Geometry: final body of the model. Coordinates: model frame, mm. A direction names the side the tool comes from. Coordinates: 2 decimals unless noted, no trailing zeros. Order: outer loops, then holes, each group sorted by start corner. A loop starts at its lowest first (then second) coordinate and runs counter-clockwise, first axis right, second up. Notation, with made-up numbers: M 74.25,56 L 94.25,56 A20 ccw 94.25,64 Z; hole C 56,0.5 d4. An arc over 180 degrees is marked long. One line per question, with ' | ' between items.
from build123d import *

# Parameters (mm, degrees)
SKETCH_1_R               = 10
EXTRUDE_1_DEPTH          = 98
CUT_EXTRUDE_1_DEPTH      = 10
CUT_EXTRUDE_1_DEPTH_BACK = 10
SKETCH_2_W               = 2.5
SKETCH_2_H               = 20
HOLE_WIZARD_M6_1_D       = 5
SKETCH_5_W               = 0.5
SKETCH_5_H               = 1.3


with BuildPart() as part:
    # 草图1 → 凸台-拉伸1 (new body)
    with BuildSketch(Plane(origin=(0, 0, 0), x_dir=(1, 0, 0), z_dir=(0, 1, 0))):
        with Locations(Location((0, 0, 0), (0, 0, 270))):
            Circle(SKETCH_1_R)
    extrude(amount=EXTRUDE_1_DEPTH)

    # 草图2 → 切除-拉伸1 (cut, two sides: drawn at the far end of the back side and taken through both)
    with BuildSketch(Plane(origin=(0, 0, 0), x_dir=(0, 0, -1), z_dir=(1, 0, 0)).offset(-CUT_EXTRUDE_1_DEPTH_BACK)):
        with Locations((8.75, 88)):
            Rectangle(SKETCH_2_W, SKETCH_2_H)
        with Locations((-8.75, 88)):
            Rectangle(SKETCH_2_W, SKETCH_2_H)
        with Locations((-8.75, 10)):
            Rectangle(SKETCH_2_W, SKETCH_2_H)
        with Locations((8.75, 10)):
            Rectangle(SKETCH_2_W, SKETCH_2_H)
    extrude(amount=CUT_EXTRUDE_1_DEPTH + CUT_EXTRUDE_1_DEPTH_BACK, mode=Mode.SUBTRACT)

    # M6 螺纹孔1 (through all)
    with Locations(Plane(origin=(10, 0, 0), x_dir=(0, 0, -1), z_dir=(1, 0, 0))):
        with Locations((0, 88), (0, 10)):
            Hole(HOLE_WIZARD_M6_1_D / 2)

    # 草图5 → 切除-旋转1 (revolve, cut)
    with BuildSketch(Plane.XY, mode=Mode.PRIVATE) as cut_revolve_1_sk:
        with Locations((-9.75, 63.65)):
            Rectangle(SKETCH_5_W, SKETCH_5_H)
        with Locations((-9.75, 34.35)):
            Rectangle(SKETCH_5_W, SKETCH_5_H)
    revolve(cut_revolve_1_sk.sketch.rotate(Axis((0, 98, 0), (0, -1, 0)), 270), axis=Axis((0, 98, 0), (0, -1, 0)), mode=Mode.SUBTRACT)


solid = part.part
1. Draft query along Y for faces 1 (the face through (0, 10, -7.5)), 2 (the face through (4, 33.7, 9)), 3 (the face through (0, 20, 8)), 4 (the face through (-0.14, 7.56, -0.54)). Return one class per face: pulls with the +Y half, pulls with the -Y half, needs draft (parallel to the pull), parting line crosses it, or undercut.
Response values:
face 1: needs draft | face 2: undercut | face 3: pulls with the -Y half | face 4: undercut
2. Section B-B, the plane x = 0. Give the number of separate pieces and of enclosed holes in the cut face, and give its area (3 significant figures).
Response values:
separate pieces: 1 | enclosed holes: 2 | area: 1,720 mm^2
3. Pin query (flat end, axial travel): P1, Ø3, axis at x = -1.5, z = 9.5, coming from the +Y side; P2, Ø4, axis at y = 11, z = 5.5, coming from the -X side; P3, Ø10.5, axis at x = -3, y = 11, coming from the +Z side; P4, Ø3, axis at y = 10, z = 0, coming from the +X side. Return the tip coordinate at first contact, or that it passes through.
Response values:
P1: stops at y = 78 | P2: stops at x = -9.37 | P3: stops at z = 7.5 | P4: passes through
4. Section C-C, the plane y = 88. Output: boundary loops of the cut face in (x, z), and give its area (3 significant figures).
Response values:
outline: M -9.68,-2.5 A10 ccw -6.61,-7.5 L 6.61,-7.5 A10 ccw 9.68,-2.5 Z; M -9.68,2.5 L 9.68,2.5 A10 ccw 6.61,7.5 L -6.61,7.5 A10 ccw Z | area: 170 mm^2
5. Material intervals for line 1 (Y direction, x = 0, z = 0); line 2 (Z direction, x = 3.5, y = 93); line 3 (Y direction, x = 0.5, z = 2.25), sorted ascending. Write a range as [from, to].
Response values:
line 1: y = [0, 7.5], [12.5, 85.5], [90.5, 98] | line 2: z = [-7.5, 7.5] | line 3: y = [0, 8.91], [11.09, 86.91], [89.09, 98]
6. Access query for faces 5 (the face through (0, 78, 8)), 6 (the face through (9.915, 20.359, -1.302)), 7 (the face through (5.78, 34.36, -7.54)), 8 (the face through (0, 88, -7.5)). Directions: +Z, -Z, +X, -X, +Y, -Y. A direction counts if a zero-diameter tool reaches every point of the face in a straight line with its end or side. Return the directions, or none.
Response values:
face 5: +Z, +X, -X, +Y | face 6: +Y, -Y | face 7: none | face 8: -Z, +X, -X, +Y
7. Section A-A, the plane z = 0. Output: boundary loops of the cut face in (x, y).
Response values:
outline: M -10,0 L 10,0 L 10,7.5 L -10,7.5 Z; M -10,12.5 L 10,12.5 L 10,33.7 L 9.5,33.7 L 9.5,35 L 10,35 L 10,63 L 9.5,63 L 9.5,64.3 L 10,64.3 L 10,85.5 L -10,85.5 L -10,64.3 L -9.5,64.3 L -9.5,63 L -10,63 L -10,35 L -9.5,35 L -9.5,33.7 L -10,33.7 Z; M -10,90.5 L 10,90.5 L 10,98 L -10,98 Z
8. Section D-D, the plane z = 6. Output: boundary loops of the cut face in (x, y).
Response values:
outline: M -8,0 L 8,0 L 8,33.7 L 7.37,33.7 L 7.37,35 L 8,35 L 8,63 L 7.37,63 L 7.37,64.3 L 8,64.3 L 8,98 L -8,98 L -8,64.3 L -7.37,64.3 L -7.37,63 L -8,63 L -8,35 L -7.37,35 L -7.37,33.7 L -8,33.7 Z
